Design review of the part built by this model. Coordinates are the model's own, in mm. Coordinates: 2 decimals unless noted, no trailing zeros. Loops run counter-clockwise (first coordinate to the right, second up) from the corner with the lowest first, then second, coordinate; pieces in that order, holes last. Notation, with made-up numbers: M 20.25,-9.5 L 24.25,-9.5 A25 ccw 24.25,8.5 Z; hole C -30.75,-7 d11. An arc over 180 degrees is marked long. Put each result on its own line as item: value. Start each with the question number.
(1) Take a section at B-B, the plane z = 10.25. Give the boundary of the cut face in (x, y).
(2) For probe 1 along Y at (x, z) = (0.25, 9.25); probe 2 along X at (y, z) = (-3.75, 10.25); probe 3 along X at (y, z) = (2, 10), list the stretches that pass through material, from the lowest coordinate up. Write a range as [from, to].
(3) Clearance check with flat-ended pins moving along their axes: pin 1 (3 mm diameter, centred on x = -7, z = 7.5, fed in from -Y); pin 2 (1.5 mm diameter, centred on x = 3.5, y = 2, fed in from +Z); pin 3 (5 mm diameter, centred on y = -8, z = 1.5, fed in from +X); pin 4 (5 mm diameter, centred on x = 3.5, z = 3.5, fed in from -Y). State where each tip first meets the part, or that it passes through.
(4) Take a section at A-A, the plane z = 8. Give the boundary of the cut face in (x, y), then the cut area to 3 significant figures.
```python
from build123d import *

# Parameters (mm, degrees)
SKETCH_1_R          = 5.188125
EXTRUDE_652_DEPTH   = 10.8
SKETCH_2_OUTSIDE_W  = 89.934
SKETCH_2_OUTSIDE_H  = 92.718
SKETCH_2_OUTSIDE_R  = 9
CUT_EXTRUDE_1_DEPTH = 18.482562741
CUT_EXTRUDE_1_DRAFT = -60
SKETCH_3_OUTSIDE_W  = 89.934
SKETCH_3_OUTSIDE_H  = 92.718
SKETCH_3_OUTSIDE_R  = 9
CUT_EXTRUDE_2_DEPTH = 18.482562741
CUT_EXTRUDE_2_DRAFT = -60
CHAMFER_1_SIZE      = 0.196428571


with BuildPart() as part:
    # 草图1 → Extrude 652 (new body)
    with BuildSketch(Plane.XY):
        Polygon((0, 10.392304845), (-9, 5.196152423), (-9, -5.196152423), (0, -10.392304845), (9, -5.196152423), (9, 5.196152423), align=None)
        with Locations(Location((0, 0, 0), (0, 0, 180))):
            Circle(SKETCH_1_R, mode=Mode.SUBTRACT)
    extrude(amount=EXTRUDE_652_DEPTH)


with BuildPart() as cut_extrude_1_tool:
    # 草图2 outside → 切除-拉伸1 (with draft: the straight prism first)
    with BuildSketch(Plane(origin=(0, 0, 0), x_dir=(-1, 0, 0), z_dir=(0, 0, -1))):
        Rectangle(SKETCH_2_OUTSIDE_W, SKETCH_2_OUTSIDE_H)
        Circle(SKETCH_2_OUTSIDE_R, mode=Mode.SUBTRACT)
    extrude(amount=-CUT_EXTRUDE_1_DEPTH)
    # 切除-拉伸1: the draft: its side faces are tilted about the plane it starts from
    cut_extrude_1_sides = [cut_extrude_1_tool.faces().sort_by_distance(p)[0] for p in [
        (0, -46.359, 9.241281371),
        (-44.967, 0, 9.241281371),
        (0, 46.359, 9.241281371),
        (44.967, 0, 9.241281371),
        (9, 0, 9.241281371),
    ]]
    draft(cut_extrude_1_sides, Plane(origin=(0, 0, 0), x_dir=(-1, 0, 0), z_dir=(0, 0, -1)), CUT_EXTRUDE_1_DRAFT)


with BuildPart() as part_1:
    add(part.part)

    # 切除-拉伸1: cut by cut_extrude_1_tool
    add(cut_extrude_1_tool.part, mode=Mode.SUBTRACT)


with BuildPart() as cut_extrude_2_tool:
    # 草图3 outside → 切除-拉伸2 (with draft: the straight prism first)
    with BuildSketch(Plane.XY.offset(10.8)):
        Rectangle(SKETCH_3_OUTSIDE_W, SKETCH_3_OUTSIDE_H)
        Circle(SKETCH_3_OUTSIDE_R, mode=Mode.SUBTRACT)
    extrude(amount=-CUT_EXTRUDE_2_DEPTH)
    # 切除-拉伸2: the draft: its side faces are tilted about the plane it starts from
    cut_extrude_2_sides = [cut_extrude_2_tool.faces().sort_by_distance(p)[0] for p in [
        (0, -46.359, 1.558718629),
        (44.967, 0, 1.558718629),
        (0, 46.359, 1.558718629),
        (-44.967, 0, 1.558718629),
        (-9, 0, 1.558718629),
    ]]
    draft(cut_extrude_2_sides, Plane.XY.offset(10.8), CUT_EXTRUDE_2_DRAFT)


with BuildPart() as part_2:
    add(part_1.part)

    # 切除-拉伸2: cut by cut_extrude_2_tool
    add(cut_extrude_2_tool.part, mode=Mode.SUBTRACT)

    # 倒角1
    chamfer_1_edges = [part_2.edges().sort_by_distance(p)[0] for p in [
        (5.188125, 0, 0),
        (5.188125, 0, 10.8),
    ]]
    chamfer(chamfer_1_edges, length=CHAMFER_1_SIZE)


solid = part_2.part
```
Computed values:
1. outline: M -9,-4.25 A9.95 ccw -8.18,-5.67 L -0.82,-9.92 A9.95 ccw 0.82,-9.92 L 8.18,-5.67 A9.95 ccw 9,-4.25 L 9,4.25 A9.95 ccw 8.18,5.67 L 0.82,9.92 A9.95 ccw -0.82,9.92 L -8.18,5.67 A9.95 ccw -9,4.25 Z; hole C 0,0 d10.38
2. probe 1: y = [-10.25, -5.18], [5.18, 10.25]
2. probe 2: x = [-9, -3.59], [3.59, 9]
2. probe 3: x = [-9, -4.79], [4.79, 9]
3. pin 1: stops at y = -7.22
3. pin 2: passes through
3. pin 3: stops at x = 8.47
3. pin 4: stops at y = -9.81
4. outline: M -9,-5.2 L 0,-10.39 L 9,-5.2 L 9,5.2 L 0,10.39 L -9,5.2 Z; hole C 0,0 d10.38
4. area: 196 mm^2
